Source: CAD feature listing. Evaluate the final solid. Frame: model axes, mm. A direction names the side the tool comes from. Coordinates: 2 decimals unless noted, no trailing zeros. Loops run counter-clockwise (first coordinate to the right, second up) from the corner with the lowest first, then second, coordinate; pieces in that order, holes last. Notation, with made-up numbers: (-17.75, 70.5) -> (8.25, 70.5) arc R31 cw to (8.25, 103.5) -> close; hole circle Ø10 at (-28, -14.5). An arc over 180 degrees is marked (long way). Answer as CSV lines item,"result".
from build123d import *

# Parameters (mm, degrees)
SKETCH_1_W      = 84
SKETCH_1_H      = 4.25
CHAMFER_1_SIZE  = 0.5
EXTRUDE_1_DEPTH = 2.5


with BuildPart() as part:
    # 草图1 → 旋转1 (revolve)
    with BuildSketch(Plane.XY, mode=Mode.PRIVATE) as revolve_1_sk:
        with Locations((42, -2.125)):
            Rectangle(SKETCH_1_W, SKETCH_1_H)
    revolve(revolve_1_sk.sketch.rotate(Axis((-1.134146341, 0, 0), (1, 0, 0)), 270), axis=Axis((-1.134146341, 0, 0), (1, 0, 0)))

    # 倒角1
    chamfer_1_edges = [part.edges().sort_by_distance(p)[0] for p in [
        (84, 0, -4.25),
    ]]
    chamfer(chamfer_1_edges, length=CHAMFER_1_SIZE)

    # 草图2 → 凸台-拉伸1 (add)
    with BuildSketch(Plane.ZY):
        with BuildLine():
            Line((-8, 6.685438565), (-8, -6))
            Line((-8, -6), (8, -6))
            Line((8, -6), (8, 6.685438565))
            ThreePointArc((8, 6.685438565), (0, 8), (-8, 6.685438565))
        make_face()
    extrude(amount=EXTRUDE_1_DEPTH)


solid = part.part
(1) Pin query (flat end, axial travel): pin 1 Ø5 at (x, y) = (72.5, 3) entering from +Z; pin 2 Ø1 at (x, z) = (47, 2.5) entering from +Y; pin 3 Ø1.5 at (x, z) = (68, -4) entering from +Y. Return the tip coordinate at first contact, or that it passes through.
Computed values:
pin 1,"z = 4.22"
pin 2,"y = 3.75"
pin 3,"y = 2.74"
(2) Cut plane B-B (y = 0). Return the cut outline in (x, z).
Computed values:
outline,"(-2.5, -8) -> (0, -8) -> (0, -4.25) -> (83.5, -4.25) -> (84, -3.75) -> (84, 3.75) -> (83.5, 4.25) -> (0, 4.25) -> (0, 8) -> (-2.5, 8) -> close"
(3) Cut plane A-A (z = 0). Return the cut outline in (x, y).
Computed values:
outline,"(-2.5, -6) -> (0, -6) -> (0, -4.25) -> (83.5, -4.25) -> (84, -3.75) -> (84, 3.75) -> (83.5, 4.25) -> (0, 4.25) -> (0, 8) -> (-2.5, 8) -> close"
(4) Cut plane C-C (x = 44). Return the cut outline in (y, z), then the cut area to 3 significant figures.
Computed values:
outline,"circle Ø8.5 at (0, 0)"
area,"56.7 mm^2"
(5) Cut plane D-D (z = -6.5). Return the cut outline in (x, y), then the cut area to 3 significant figures.
Computed values:
outline,"(-2.5, -6) -> (0, -6) -> (0, 7.14) -> (-2.5, 7.14) -> close"
area,"32.9 mm^2"
(6) Material intervals for L1, parallel to X at y = -3, z = 5; L2, parallel to Y at x = 70.5, z = -3; L3, parallel to Z at x = 41.5, y = 3.75, sorted ascending. Write a range as [from, to].
Computed values:
L1,"[-2.5, 0]"
L2,"[-3.01, 3.01]"
L3,"[-2, 2]"
(7) Access query for faces 1 (the flat face through (84, 0, 0)), 2 (the flat face through (0, 4, -2)). Directions: +Z, -Z, +X, -X, +Y, -Y. A direction counts if a zero-diameter tool reaches every point of the face in a straight line with its end or side. Return the directions, or none.
Computed values:
face 1,"+Z, -Z, +X, +Y, -Y"
face 2,"+X"
